Source: CAD feature listing. Evaluate the final solid. Frame: model axes, mm. A direction names the side the tool comes from. Round coordinates to 2 decimals unless told otherwise and drop trailing zeros. Loops run counter-clockwise (first coordinate to the right, second up) from the corner with the lowest first, then second, coordinate; pieces in that order, holes last. Notation, with made-up numbers: (79.5, 5.5) - (127.5, 5.5) arc R18 ccw to (127.5, 25.5) - close; hole circle Ø11 at (10, -22.75). An arc over 180 degrees is marked (long way). One line per question, with ' | ' between items.
from build123d import *

# Parameters (mm, degrees)
SKETCH1_R           = 27.5
SKETCH1_R_2         = 20
BOSS_EXTRUDE1_DEPTH = 15
CUT_EXTRUDE1_START  = -5
SKETCH2_R           = 27.5
SKETCH2_R_2         = 22.5
CUT_EXTRUDE1_DEPTH  = 5
CHAMFER1_SIZE       = 1


with BuildPart() as part:
    # Sketch1 → Boss-Extrude1 (new body)
    with BuildSketch(Plane.XY):
        Circle(SKETCH1_R)
        Circle(SKETCH1_R_2, mode=Mode.SUBTRACT)
    extrude(amount=BOSS_EXTRUDE1_DEPTH)

    # Sketch2 → Cut-Extrude1 (cut)
    with BuildSketch(Plane.XY.offset(15).offset(CUT_EXTRUDE1_START)):
        Circle(SKETCH2_R)
        Circle(SKETCH2_R_2, mode=Mode.SUBTRACT)
    extrude(amount=CUT_EXTRUDE1_DEPTH, mode=Mode.SUBTRACT)

    # Chamfer1
    chamfer1_edges = [part.edges().sort_by_distance(p)[0] for p in [
        (-27.5, 0, 10),
        (-22.5, 0, 15),
        (-27.5, 0, 0),
        (-20, 0, 0),
    ]]
    chamfer(chamfer1_edges, length=CHAMFER1_SIZE)


solid = part.part
1. Section query A-A, the plane y = 0. Return loops of the section in (x, z), plus the area to 3 significant figures.
Worked out:
outline: (-27.5, 1) - (-26.5, 0) - (-21, 0) - (-20, 1) - (-20, 15) - (-21.5, 15) - (-22.5, 14) - (-22.5, 10) - (-26.5, 10) - (-27.5, 9) - close; (20, 1) - (21, 0) - (26.5, 0) - (27.5, 1) - (27.5, 9) - (26.5, 10) - (22.5, 10) - (22.5, 14) - (21.5, 15) - (20, 15) - close | area: 171 mm2
2. Access query for faces 1 (the flat face through (16, -13, 15)), 2 (the flat face through (-12, -20, 10)). Directions: +Z, -Z, +X, -X, +Y, -Y. A direction counts if a zero-diameter tool reaches every point of the face in a straight line with its end or side. Return the directions, or none.
Worked out:
face 1: +Z, +X, -X, +Y, -Y | face 2: +Z
3. Material intervals for probe 1 along Y at (x, z) = (0, 6); probe 2 along Z at (x, y) = (23, -6); probe 3 along Y at (x, z) = (-8, 12), sorted ascending.
Worked out:
probe 1: y = -27.5 to -20, 20 to 27.5 | probe 2: z = 0 to 10 | probe 3: y = -21.03 to -18.33, 18.33 to 21.03
4. Mould query, pull axis X, two halves, no side actions, for faces 3 (the cylindrical face through (-4.336, -19.524, 7.902)), 4 (the flat face through (-16, 14, 0)), 5 (the cylindrical face through (-5.961, -26.846, 4.944)). Classes: released by +X, released by -X, zero draft, split by the parting line, or undercut.
Worked out:
face 3: undercut | face 4: zero draft | face 5: split by the parting line
5. Contact query for flat-ended pins moving along their axis: P1, Ø4, axis at y = 19, z = 6, coming from the -X side; P2, Ø2, axis at x = -20, z = 9.5, coming from the +Y side; P3, Ø8, axis at x = 6.5, z = 4.5, coming from the -Y side. Output: stop coordinate, or through.
Worked out:
P1: stops at x = -21.62 | P2: stops at y = 19.75 | P3: stops at y = -27.39
6. Section query C-C, the plane z = 5.5. Return loops of the section in (x, y).
Worked out:
outline: circle Ø55 at (0, 0); hole circle Ø40 at (0, 0)
